from build123d import *

# Parameters (mm, degrees)
BRACKET_BODY_DEPTH      = 75
FLANGE_A_HOLES_SKETCH_R = 6
FLANGE_A_HOLES_2X_DEPTH = 75
FLANGE_B_HOLES_SKETCH_R = 6
FLANGE_B_HOLES_2X_DEPTH = 75
PIVOT_BORE_SKETCH_R     = 12.5
PIVOT_BORE_DEPTH        = 75


with BuildPart() as part:
    # Bracket Profile Sketch → Bracket Body (new body)
    with BuildSketch(Plane.XY):
        with BuildLine():
            Line((0, -25), (60, -25))
            ThreePointArc((60, -25), (68.485281374, -21.485281374), (72, -13))
            Line((72, -13), (72, 57))
            Line((72, 57), (56, 57))
            Line((56, 57), (56, -3))
            ThreePointArc((56, -3), (54.242640687, -7.242640687), (50, -9))
            Line((50, -9), (23.323807579, -9))
            ThreePointArc((23.323807579, -9), (20.615528128, 14.142135624), (0, 25))
            Line((0, 25), (-48, 25))
            Line((-48, 25), (-48, 9))
            Line((-48, 9), (-23.323807579, 9))
            ThreePointArc((-23.323807579, 9), (-20.615528128, -14.142135624), (0, -25))
        make_face()
    extrude(amount=BRACKET_BODY_DEPTH)

    # Flange A Holes Sketch → Flange A Holes 2x (cut)
    with BuildSketch(Plane(origin=(0, 25, 0), x_dir=(1, 0, 0), z_dir=(0, 1, 0))):
        with Locations(Location((-32, -15.5, 0), (0, 0, 270))):
            Circle(FLANGE_A_HOLES_SKETCH_R)
        with Locations(Location((-32, -59.5, 0), (0, 0, 270))):
            Circle(FLANGE_A_HOLES_SKETCH_R)
    extrude(amount=-FLANGE_A_HOLES_2X_DEPTH, mode=Mode.SUBTRACT)

    # Flange B Holes Sketch → Flange B Holes 2x (cut)
    with BuildSketch(Plane(origin=(72, 0, 0), x_dir=(0, 0, -1), z_dir=(1, 0, 0))):
        with Locations((-59, 41)):
            Circle(FLANGE_B_HOLES_SKETCH_R)
        with Locations((-16, 41)):
            Circle(FLANGE_B_HOLES_SKETCH_R)
    extrude(amount=-FLANGE_B_HOLES_2X_DEPTH, mode=Mode.SUBTRACT)

    # Pivot Bore Sketch → Pivot Bore (cut)
    with BuildSketch(Plane.XY.offset(75)):
        Circle(PIVOT_BORE_SKETCH_R)
    extrude(amount=-PIVOT_BORE_DEPTH, mode=Mode.SUBTRACT)


solid = part.part
Model file for the job. Use its own axes, mm. A direction names the side the tool comes from. Give positions to 0.01 mm unless a question says otherwise; leave off trailing zeros. Order: outer loops, then holes, each group sorted by start corner. A loop starts at its lowest first (then second) coordinate and runs counter-clockwise, first axis right, second up. Notation, with made-up numbers: (54.5, -27.5) -> (64.5, -27.5) arc R18 ccw to (64.5, -10.5) -> close; hole circle Ø10 at (35, 50.25). An arc over 180 degrees is marked (long way). Use CSV: the item, a comma, the result in double quotes.
1. Band-saw the part on B-B, the plane x = -32. Give the cut face in (y, z), then the cut area to 3 significant figures.
Outcome:
outline,"(9, 0) -> (25, 0) -> (25, 9.5) -> (9, 9.5) -> close; (9, 21.5) -> (25, 21.5) -> (25, 53.5) -> (9, 53.5) -> close; (9, 65.5) -> (25, 65.5) -> (25, 75) -> (9, 75) -> close"
area,"816 mm²"
2. Drop flat-ended pins along their axis: pin 1 (19 mm diameter, centred on x = -32, z = 15.5, fed in from -Y); pin 2 (12 mm diameter, centred on x = 5.5, z = 37.5, fed in from +Y); pin 3 (7.5 mm diameter, centred on x = -36.5, z = 23.5, fed in from -Y); pin 4 (9.5 mm diameter, centred on y = 41, z = 16, fed in from +X). Give the stop position or say it passes through.
Outcome:
pin 1,"y = -10.9"
pin 2,"y = 25"
pin 3,"y = 9"
pin 4,"through"
3. Band-saw the part on C-C, the plane y = 41. Give the cut face in (x, z), then the cut area to 3 significant figures.
Outcome:
outline,"(56, 0) -> (72, 0) -> (72, 10) -> (56, 10) -> close; (56, 22) -> (72, 22) -> (72, 53) -> (56, 53) -> close; (56, 65) -> (72, 65) -> (72, 75) -> (56, 75) -> close"
area,"816 mm²"
4. Band-saw the part on D-D, the plane z = 68. Give the cut face in (x, y).
Outcome:
outline,"(-48, 9) -> (-23.32, 9) arc R25 ccw to (0, -25) -> (60, -25) arc R12 ccw to (72, -13) -> (72, 57) -> (56, 57) -> (56, -3) arc R6 cw to (50, -9) -> (23.32, -9) arc R25 ccw to (0, 25) -> (-48, 25) -> close; hole circle Ø25 at (0, 0)"
5. Drill centre lines: line 1 along Z through (x, y) = (61, 43); line 2 along X through (y, z) = (47, 71); line 3 along X through (y, z) = (20, 59.5). Where is each one in solid material? Low to high. Write a range as from..to.
Outcome:
line 1,"0..10.34, 21.66..53.34, 64.66..75"
line 2,"56..72"
line 3,"-48..-38, -26..15, 56..72"
6. 3-axis set-ups, long thin cutter, end or side, ignore diameter. For faces 5 (the flat face through (21, 1, 0)), 6 (the flat face through (56, 27, 37)): which of +Z, -Z, +X, -X, +Y, -Y reach the whole face in a straight line?
Outcome:
face 5,"-Z, +X, -X, +Y, -Y"
face 6,"+Z, -Z, +Y"
7. Band-saw the part on A-A, the plane z = 19. Give the cut face in (x, y).
Outcome:
outline,"(-48, 9) -> (-36.87, 9) -> (-36.87, 25) -> (-48, 25) -> close; (-27.13, 9) -> (-23.32, 9) arc R25 ccw to (0, -25) -> (60, -25) arc R12 ccw to (72, -13) -> (72, 35.8) -> (56, 35.8) -> (56, -3) arc R6 cw to (50, -9) -> (23.32, -9) arc R25 ccw to (0, 25) -> (-27.13, 25) -> close; (56, 46.2) -> (72, 46.2) -> (72, 57) -> (56, 57) -> close; hole circle Ø25 at (0, 0)"
8. Mould opens along X. For faces 1 (the cylindrical face through (68.39, -21.58, 36.98)), 2 (the cylindrical face through (54.289, -7.196, 36.975)), 3 (the flat face through (21, 1, 75)), 4 (the cylindrical face through (-35.65, 17.11, 54.74)) say: +X half, -X half, draft (parallel to the pull), parting line (faces both ways), or undercut.
Outcome:
face 1,"+X half"
face 2,"undercut"
face 3,"draft"
face 4,"undercut"
